```python
from build123d import *


with BuildPart() as part:
    # Sketch1 → Revolve1 (revolve)
    with BuildSketch(Plane.XY, mode=Mode.PRIVATE) as revolve1_sk:
        Polygon((-29.5, 0), (-65, 0), (-65, 25), (-40, 25), (-40, 50), (-27.5, 50), (-27.5, 2), align=None)
    revolve(revolve1_sk.sketch.rotate(Axis((0, 0, 0), (0, 1, 0)), 270), axis=Axis((0, 0, 0), (0, 1, 0)))


solid = part.part
```
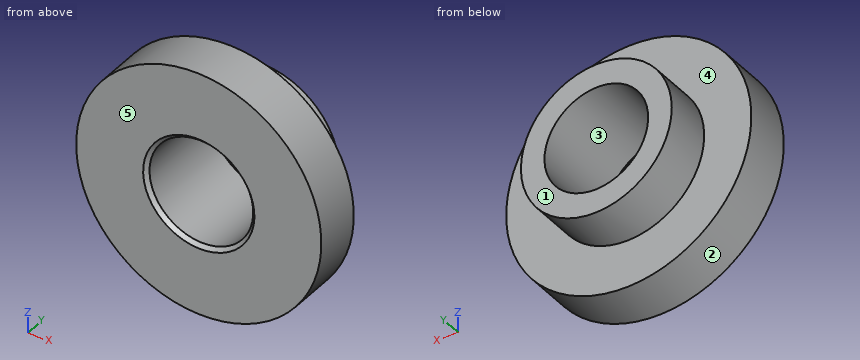
The listing builds one solid part. Answer for the finished solid, in the listing's coordinates (mm). Face numbers are marked on the shaded views. A direction names the side the tool comes from. Give positions to 0.01 mm unless a question says otherwise; leave off trailing zeros. Loops run counter-clockwise (first coordinate to the right, second up) from the corner with the lowest first, then second, coordinate; pieces in that order, holes last. Notation, with made-up numbers: (-14.5, 43.5) - (0.5, 43.5) arc R27 cw to (0.5, 64.5) - close; hole circle Ø3 at (59, 79). An arc over 180 degrees is marked (long way). Return JSON: item names as keys, results as strings. Group by question number.
1. Find section A-A (z = 0). Write down the section's boundary in (x, y), then the cut area to 3 significant figures.
2. Straight lines are drawn through the part: line 1 (X direction, y = 21.5, z = 0); line 2 (X direction, y = 40, z = 0); line 3 (Y direction, x = 40, z = 39). For each, find the intervals that lie inside material, in ascending order. Write a range as [from, to].
3. Find section D-D (z = -33). Write down the section's boundary in (x, y), then the cut area to 3 significant figures.
4. Find section B-B (x = 0). Write down the section's boundary in (y, z).
5. Which of the six approach directions +Z, -Z, +X, -X, +Y, -Y give full straight-line access (tool end or side, diameter ignored) to the marked faces 4 and 5?
6. Determine the mould class of the marked faces 1, 2 and 3 for opening direction Z: pulls with the +Z half, pulls with the -Z half, needs draft (parallel to the pull), parting line crosses it, or undercut.
7. Given pin 1 Ø4 at (y, z) = (42, 18.5) entering from -X; pin 2 Ø3 at (x, y) = (15.5, 23.5) entering from +Z; pin 3 Ø12 at (y, z) = (11, 20.5) entering from +X, each flat-ended and moving along its own axis, determine where each tip first touches the part or whether it passes through.
8. Find section C-C (y = 31). Write down the section's boundary in (x, z), then the cut area to 3 significant figures.
Verdict:
{
 "1": {"outline": "(-65, 0) - (-29.5, 0) - (-27.5, 2) - (-27.5, 50) - (-40, 50) - (-40, 25) - (-65, 25) - close; (27.5, 2) - (29.5, 0) - (65, 0) - (65, 25) - (40, 25) - (40, 50) - (27.5, 50) - close", "area": "2,500 mm^2"},
 "2": {"line 1": "x = [-65, -27.5], [27.5, 65]", "line 2": "x = [-40, -27.5], [27.5, 40]", "line 3": "y = [0, 25]"},
 "3": {"outline": "(-56, 0) - (56, 0) - (56, 25) - (22.61, 25) - (22.61, 50) - (-22.61, 50) - (-22.61, 25) - (-56, 25) - close", "area": "3,930 mm^2"},
 "4": {"outline": "(0, -65) - (25, -65) - (25, -40) - (50, -40) - (50, -27.5) - (2, -27.5) - (0, -29.5) - close; (0, 29.5) - (2, 27.5) - (50, 27.5) - (50, 40) - (25, 40) - (25, 65) - (0, 65) - close"},
 "5": {"face 4": "+Y", "face 5": "+Z, -Z, +X, -X, -Y"},
 "6": {"face 1": "needs draft", "face 2": "parting line crosses it", "face 3": "undercut"},
 "7": {"pin 1": "stops at x = -36.44", "pin 2": "stops at z = 63.47", "pin 3": "stops at x = 63.36"},
 "8": {"outline": "circle Ø80 at (0, 0); hole circle Ø55 at (0, 0)", "area": "2,650 mm^2"}
}
